Check sheet for the drawn part. Datum: minimum x, y, z corner. Units: mm. Coordinates: 2 decimals unless noted, no trailing zeros. Write each loop counter-clockwise with the first axis right and the second up, starting at its lowest first coordinate (ties: lowest second). Pieces come first, ordered by that corner, then holes. Notation, with made-up numbers: (61.5, 30.25) -> (79.5, 30.25) arc R16 cw to (79.5, 50.25) -> close; hole circle Ø5 at (-3, 19.5). An arc over 180 degrees is marked (long way). Write item = value, one per line. Start each with the question number.
(1) Material ranges on probe 1 along X at (y, z) = (5, 5); probe 2 along Z at (x, y) = (7.1, 5), recorded low to high. Write a range as [from, to].
(2) Section check A-A (z = 3). Record the cut outline in (x, y).
(3) Section check C-C (y = 7.75). Record the cut outline in (x, z).
(4) Mould release check, pull along X, two halves, no side actions. Record for the marked faces 1, 2 and 3: released by +X, released by -X, zero draft, split by the parting line, or undercut.
(5) Section check D-D (z = 1.2). Record the cut outline in (x, y), plus the area to 3 significant figures.
(6) Section check B-B (x = 5). Record the cut outline in (y, z).
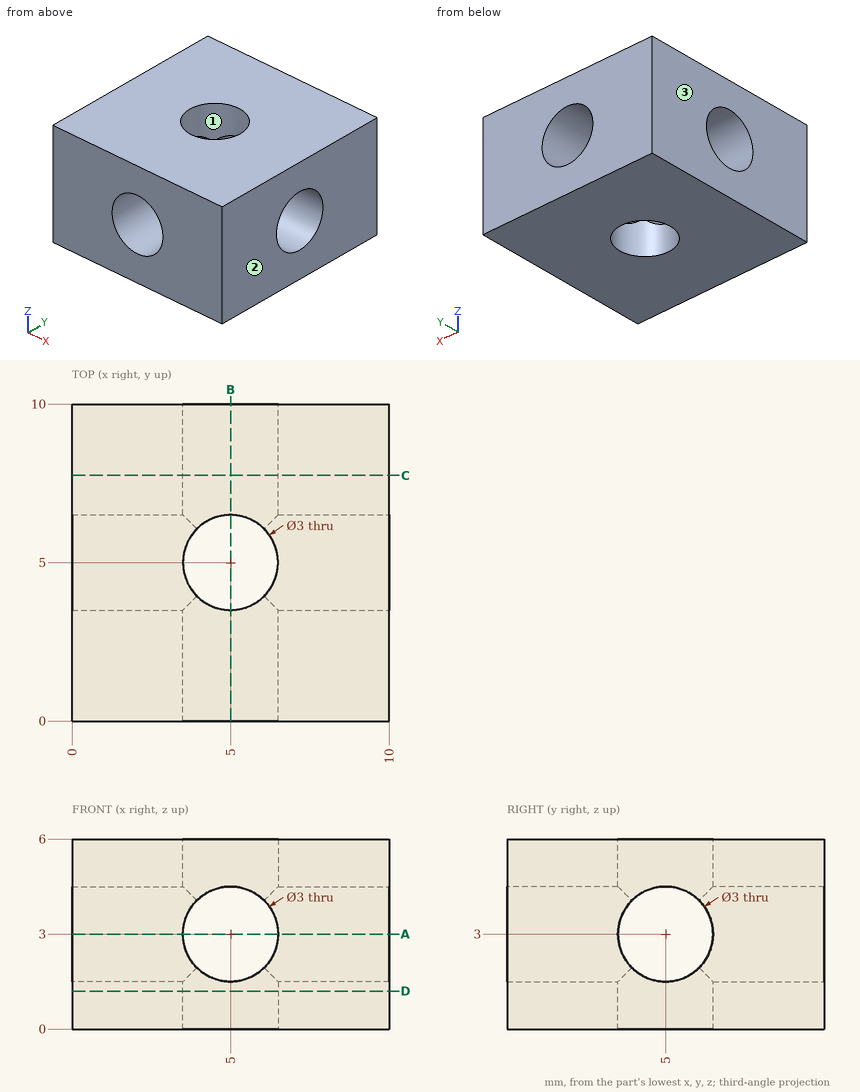
Response:
q1.probe_1 = [0, 3.5], [6.5, 10]
q1.probe_2 = [0, 1.5], [4.5, 6]
q2.outline = (0, 0) -> (3.5, 0) -> (3.5, 3.5) -> (0, 3.5) -> close; (0, 6.5) -> (3.5, 6.5) -> (3.5, 10) -> (0, 10) -> close; (6.5, 0) -> (10, 0) -> (10, 3.5) -> (6.5, 3.5) -> close; (6.5, 6.5) -> (10, 6.5) -> (10, 10) -> (6.5, 10) -> close
q3.outline = (0, 0) -> (10, 0) -> (10, 6) -> (0, 6) -> close; hole circle Ø3 at (5, 3)
q4.face_1 = undercut
q4.face_2 = released by +X
q4.face_3 = released by -X
q5.outline = (0, 0) -> (10, 0) -> (10, 10) -> (0, 10) -> close; hole circle Ø3 at (5, 5)
q5.area = 92.9 mm2
q6.outline = (0, 0) -> (3.5, 0) -> (3.5, 1.5) -> (0, 1.5) -> close; (0, 4.5) -> (3.5, 4.5) -> (3.5, 6) -> (0, 6) -> close; (6.5, 0) -> (10, 0) -> (10, 1.5) -> (6.5, 1.5) -> close; (6.5, 4.5) -> (10, 4.5) -> (10, 6) -> (6.5, 6) -> close
